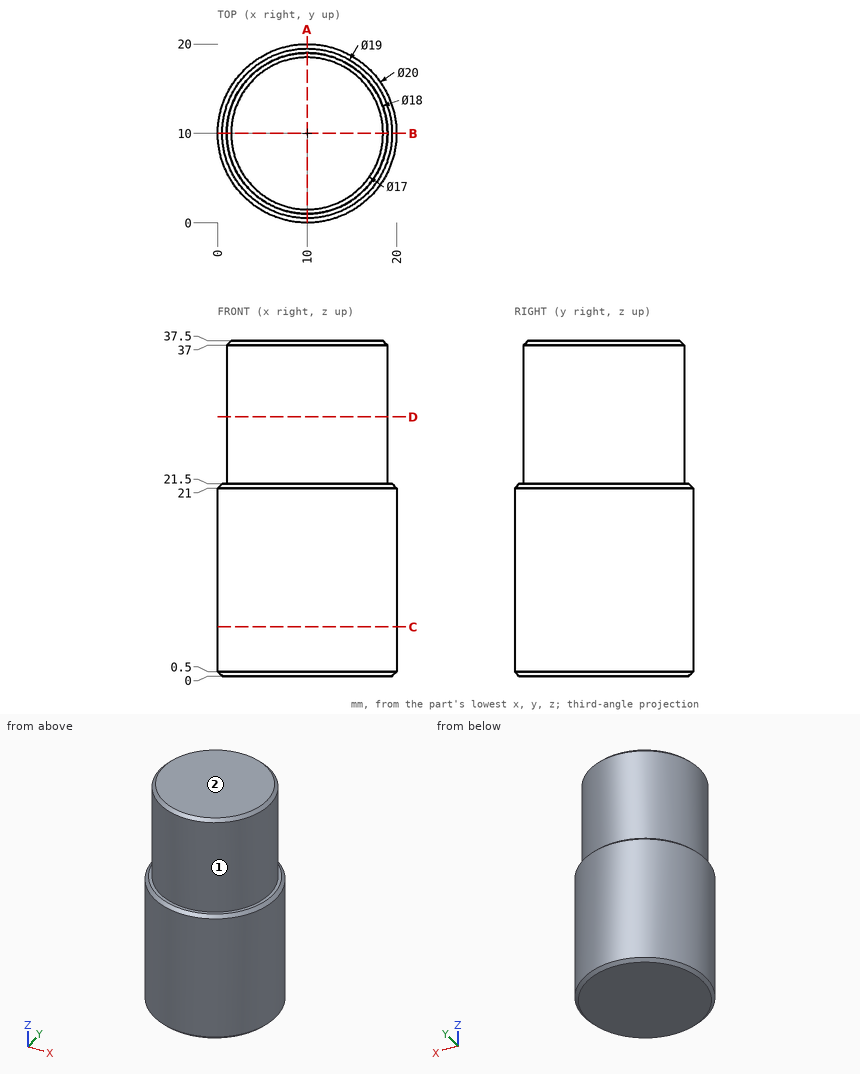
Part print with two shaded views. Sizes in mm from the minimum x, y, z corner. A direction names the side the tool comes from. Round coordinates to 2 decimals unless told otherwise and drop trailing zeros. Order: outer loops, then holes, each group sorted by start corner. A loop starts at its lowest first (then second) coordinate and runs counter-clockwise, first axis right, second up. Notation, with made-up numbers: (17, 80.25) - (60, 80.25) arc R19 cw to (60, 105.25) - close; hole circle Ø4 at (-10.75, 43.5). An arc over 180 degrees is marked (long way). Answer as CSV lines item,"result". Start each with the question number.
1. Saw through at A-A, the plane x = 10. Write the cut outline in (y, z), and give its area (3 significant figures).
2. Saw through at C-C, the plane z = 5.5. Write the cut outline in (x, y), and give its area (3 significant figures).
3. Saw through at D-D, the plane z = 29. Write the cut outline in (x, y).
4. Tool access for the marked faces 1 and 2: list every direction of +Z, -Z, +X, -X, +Y, -Y with a clear straight run to the whole face (end or side of a thin tool).
5. Pin check, flat tips, straight feed: pin 1 (10 mm diameter, centred on x = 4.5, z = 10.5, fed in from +Y); pin 2 (2 mm diameter, centred on x = 14.5, z = 9.5, fed in from -Y); pin 3 (6 mm diameter, centred on x = 15.5, z = 7, fed in from -Y). Stop position of each tip, or through.
6. Drill centre lines: L1, parallel to Z at x = 18.25, y = 14; L2, parallel to X at y = 10.25, z = 13; L3, parallel to Y at x = 17.25, z = 14. Where is each one in solid material? Low to high. Write a range as [from, to].
Model answer:
1,outline,"(0, 0.5) - (0.5, 0) - (19.5, 0) - (20, 0.5) - (20, 21) - (19.5, 21.5) - (19, 21.5) - (19, 37) - (18.5, 37.5) - (1.5, 37.5) - (1, 37) - (1, 21.5) - (0.5, 21.5) - (0, 21) - close"
1,area,"717 mm²"
2,outline,"circle Ø20 at (10, 10)"
2,area,"314 mm²"
3,outline,"circle Ø18 at (10, 10)"
4,face 1,"+Z"
4,face 2,"+Z, +X, -X, +Y, -Y"
5,pin 1,"stops at y = 19.99"
5,pin 2,"stops at y = 0.63"
5,pin 3,"stops at y = 0.32"
6,L1,"z = [0, 21.5]"
6,L2,"x = [0, 20]"
6,L3,"y = [3.11, 16.89]"
